```python
from build123d import *

# Parameters (mm, degrees)
EXTRUDE_1_DEPTH         = 4
CUT_EXTRUDE_1_REACH     = 68.408
SKETCH_2_R              = 2
CUT_EXTRUDE_2_REACH     = 68.408
SKETCH_3_R              = 2.1
HOLE_WIZARD_M2_1_REACH  = 86.054
HOLE_WIZARD_M2_1_BORE_R = 0.8
CUT_EXTRUDE_3_REACH     = 60.577
CUT_EXTRUDE_4_DEPTH     = 5
FILLET_1_R              = 3
CHAMFER_1_SIZE          = 3


with BuildPart() as part:
    # 草图1 → 凸台-拉伸1 (new, symmetric)
    with BuildSketch(Plane.XY):
        Polygon((0, 0), (0, 14.5), (55, 14.5), (55, 18.5), (-25, 18.5), (-25, -18.5), (55, -18.5), (55, -14.5), (0, -14.5), align=None)
    extrude(amount=EXTRUDE_1_DEPTH, both=True)

    # 切除-拉伸1: up to this face of the body (flat: up to its plane)
    cut_extrude_1_end = Plane(part.part.faces().sort_by_distance((15, -18.5, 0))[0])
    # 草图2 → 切除-拉伸1 (cut, up to the picked face)
    with BuildSketch(Plane(origin=(0, 18.5, 0), x_dir=(1, 0, 0), z_dir=(0, 1, 0)), mode=Mode.PRIVATE) as cut_extrude_1_sk1:
        with Locations(Location((51, 0, 0), (0, 0, 180))):
            Circle(SKETCH_2_R)
    cut_extrude_1_tool1 = split(extrude(cut_extrude_1_sk1.sketch, amount=-CUT_EXTRUDE_1_REACH, mode=Mode.PRIVATE), bisect_by=cut_extrude_1_end, keep=Keep.BOTH, mode=Mode.PRIVATE)
    add(cut_extrude_1_tool1.solids().sort_by(Axis((51, 18.5, 0), (0, -1, 0)))[0], mode=Mode.SUBTRACT)

    # 草图3 → 切除-拉伸2 (cut, up to next)
    with BuildSketch(Plane.XZ.offset(18.5), mode=Mode.PRIVATE) as cut_extrude_2_sk1:
        with Locations(Location((-4, 0, 0), (0, 0, 270))):
            Circle(SKETCH_3_R)
    cut_extrude_2_tool1 = extrude(cut_extrude_2_sk1.sketch, amount=-CUT_EXTRUDE_2_REACH, mode=Mode.PRIVATE) & part.part
    add(cut_extrude_2_tool1.solids().sort_by_distance((-4, -18.5, 0))[0], mode=Mode.SUBTRACT)

    # M2 螺纹孔1 bore (on position points) → M2 螺纹孔1 (cut, up to next)
    with BuildSketch(Plane(origin=(51, -16.5, 4), x_dir=(1, 0, 0), z_dir=(0, 0, 1)), mode=Mode.PRIVATE) as hole_wizard_m2_1_sk1:
        Circle(HOLE_WIZARD_M2_1_BORE_R)
    hole_wizard_m2_1_tool1 = extrude(hole_wizard_m2_1_sk1.sketch, amount=-HOLE_WIZARD_M2_1_REACH, mode=Mode.PRIVATE) & part.part
    hole_wizard_m2_1 = hole_wizard_m2_1_tool1.solids().sort_by_distance((51, -16.5, 4))[0]
    add(hole_wizard_m2_1, mode=Mode.SUBTRACT)

    # 镜向1: M2 螺纹孔1 across plane
    add(hole_wizard_m2_1.mirror(Plane.ZX), mode=Mode.SUBTRACT)

    # 草图5 → 切除-拉伸3 (cut, up to next)
    with BuildSketch(Plane.XY.offset(4), mode=Mode.PRIVATE) as cut_extrude_3_sk1:
        with BuildLine():
            Line((-25, 4.5), (-14, 4.5))
            ThreePointArc((-14, 4.5), (-9.5, 0), (-14, -4.5))
            Line((-14, -4.5), (-25, -4.5))
            Line((-25, -4.5), (-25, 4.5))
        make_face()
    cut_extrude_3_tool1 = extrude(cut_extrude_3_sk1.sketch, amount=-CUT_EXTRUDE_3_REACH, mode=Mode.PRIVATE) & part.part
    add(cut_extrude_3_tool1.solids().sort_by_distance((-17.698151, 0, 4))[0], mode=Mode.SUBTRACT)

    # 草图6 → 切除-拉伸4 (cut)
    with BuildSketch(Plane(origin=(0, 0, -4), x_dir=(-1, 0, 0), z_dir=(0, 0, -1))):
        with BuildLine():
            Line((25, -6.5), (25, 6.5))
            Line((25, 6.5), (14, 6.5))
            ThreePointArc((14, 6.5), (7.5, 0), (14, -6.5))
            Line((14, -6.5), (25, -6.5))
        make_face()
    extrude(amount=-CUT_EXTRUDE_4_DEPTH, mode=Mode.SUBTRACT)

    # 圆角1
    fillet_1_edges = [part.edges().sort_by_distance(p)[0] for p in [
        (0, -14.5, 0),
        (0, 14.5, 0),
    ]]
    fillet(fillet_1_edges, radius=FILLET_1_R)

    # 倒角1
    chamfer_1_edges = [part.edges().sort_by_distance(p)[0] for p in [
        (-25, -18.5, 0),
        (-25, 18.5, 0),
    ]]
    chamfer(chamfer_1_edges, length=CHAMFER_1_SIZE)


solid = part.part
```
Could you check a few things on this model? Use its own coordinates, in mm. A direction names the side the tool comes from. Round coordinates to 2 decimals unless told otherwise and drop trailing zeros. Loops run counter-clockwise (first coordinate to the right, second up) from the corner with the lowest first, then second, coordinate; pieces in that order, holes last. Notation, with made-up numbers: (64, 75.25) -> (92, 75.25) arc R20 cw to (92, 110.25) -> close; hole circle Ø9 at (85, 46.5). An arc over 180 degrees is marked (long way). Put each result on its own line as item: value.
Q1. I want a section at A-A on y = 0. Write out the boundary of the cut face in (x, z), and give its area (3 significant figures).
Checks:
outline: (-9.5, 1) -> (-7.5, 1) -> (-7.5, -4) -> (0, -4) -> (0, 4) -> (-9.5, 4) -> close; hole circle Ø4.2 at (-4, 0)
area: 52.1 mm2
Q2. For pin 1 Ø3.5 at (x, z) = (-4, 0) entering from +Y; pin 2 Ø4 at (y, z) = (-4, 1.5) entering from +X; pin 3 Ø4 at (x, y) = (-14, 3) entering from -Z, each with a flat end and sliding along its axis, tell me the tip position at first contact or that it passes through.
Checks:
pin 1: through
pin 2: x = 0
pin 3: z = 1
Q3. I want a section at C-C on x = -4. Write out the boundary of the cut face in (y, z).
Checks:
outline: (-18.5, -4) -> (18.5, -4) -> (18.5, -2.1) -> (-18.5, -2.1) -> close; (-18.5, 2.1) -> (18.5, 2.1) -> (18.5, 4) -> (-18.5, 4) -> close
Q4. Which directions (+Z, -Z, +X, -X, +Y, -Y) give clear straight access to the entire face, cutting with the end or side of a thin tool? Please do faces 4 (the flat face through (-19, -6.5, -2)), 5 (the flat face through (0, 0, 0)), 6 (the flat face through (55, -17, 0)), 7 (the cylindrical face through (51.763, -16.26, 2.932)).
Checks:
face 4: -Z, -X
face 5: +Z, -Z, +X
face 6: +Z, -Z, +X, +Y, -Y
face 7: +Z
Q5. I want a section at D-D on y = 16.5. Write out the boundary of the cut face in (x, z).
Checks:
outline: (-24, -4) -> (55, -4) -> (55, 4) -> (51.8, 4) -> (51.8, 1.83) arc R2 cw (long way) to (50.2, 1.83) -> (50.2, 4) -> (-24, 4) -> close; hole circle Ø4.2 at (-4, 0)
Q6. I want a section at B-B on x = 51. Write out the boundary of the cut face in (y, z).
Checks:
outline: (-18.5, -4) -> (-14.5, -4) -> (-14.5, -2) -> (-18.5, -2) -> close; (-18.5, 2) -> (-17.3, 2) -> (-17.3, 4) -> (-18.5, 4) -> close; (-15.7, 2) -> (-14.5, 2) -> (-14.5, 4) -> (-15.7, 4) -> close; (14.5, -4) -> (18.5, -4) -> (18.5, -2) -> (14.5, -2) -> close; (14.5, 2) -> (15.7, 2) -> (15.7, 4) -> (14.5, 4) -> close; (17.3, 2) -> (18.5, 2) -> (18.5, 4) -> (17.3, 4) -> close
Q7. Thinking about a two-plate mould opening in Z: for faces 1 (the flat face through (-3, 0, 4)), 2 (the cylindrical face through (51, -16, -2)), 3 (the flat face through (-23.5, 17, -0.1)), which applies, pulls with the +Z half, pulls with the -Z half, needs draft (parallel to the pull), parting line crosses it, or undercut?
Checks:
face 1: pulls with the +Z half
face 2: undercut
face 3: needs draft
Q8. Please list where these lines run through material, in increasing order: line 1 (Y direction, x = 51, z = 2.6); line 2 (Y direction, x = 17.5, z = -1); line 3 (Z direction, x = 51, y = -16). Write a range as from..to.
Checks:
line 1: -18.5..-17.3, -15.7..-14.5, 14.5..15.7, 17.3..18.5
line 2: -18.5..-14.5, 14.5..18.5
line 3: -4..-2
